The figure shows three views and two pictorial views of one solid part (mm, origin at its lowest corner). Answer the questions. A direction names the side the tool comes from. Coordinates: 2 decimals unless noted, no trailing zeros. Loops run counter-clockwise (first coordinate to the right, second up) from the corner with the lowest first, then second, coordinate; pieces in that order, holes last.
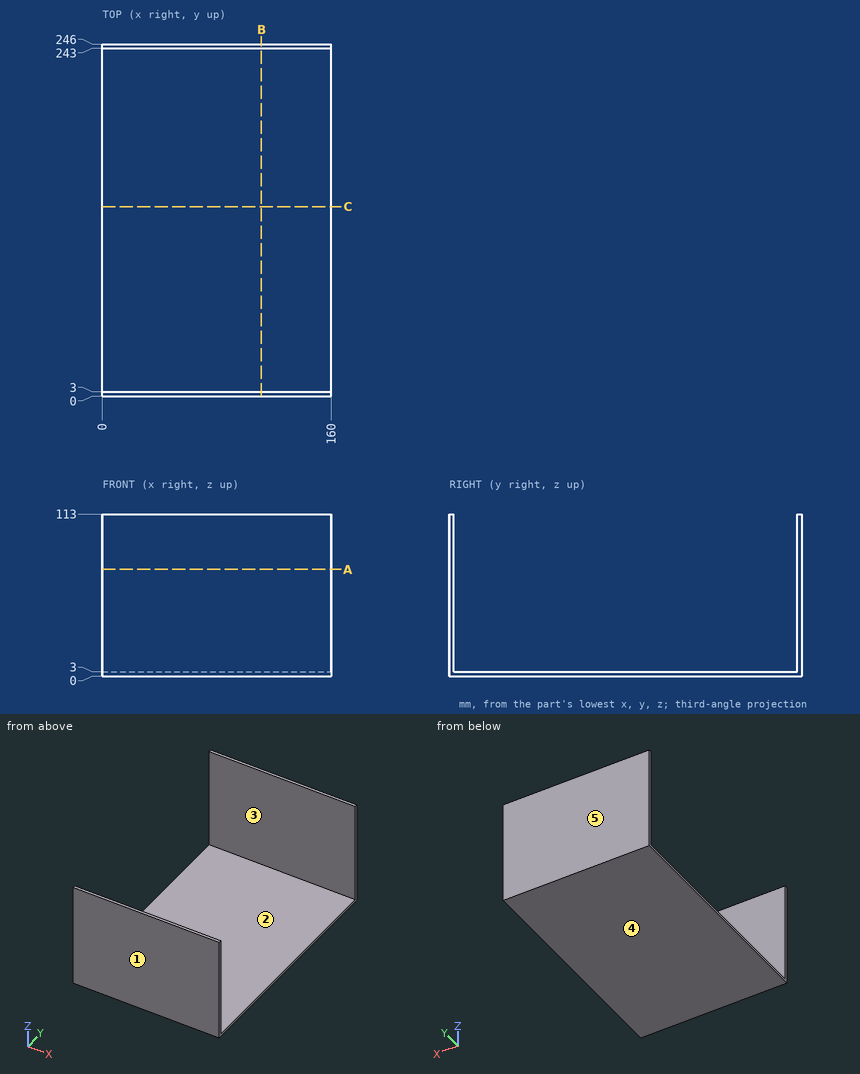
1. For the marked faces 1 and 2, determine the directions among +Z, -Z, +X, -X, +Y, -Y from which every point of the face is accessible in a straight line to the end or side of a thin tool.
2. A cutting plane is placed at A-A, the plane z = 74.5. Give the vertices of the cut face in (x, y), then the cut area to 3 significant figures.
3. Each of these flat-tipped pins is pushed along its axis until it touches: P1, Ø3, axis at x = 113, z = 70, coming from the -Y side; P2, Ø1, axis at x = 87.5, y = 116, coming from the +Z side. Where does it stop, or does it pass through?
4. A cutting plane is placed at C-C, the plane y = 132.5. Give the vertices of the cut face in (x, z).
5. Determine the mould class of the marked faces 3, 4 and 5 for opening direction Y: released by +Y, released by -Y, zero draft, split by the parting line, or undercut.
6. A cutting plane is placed at B-B, the plane x = 111. Give the vertices of the cut face in (y, z), then the cut area to 3 significant figures.
7. Straight lines are drawn through the part: probe 1 along Y at (x, z) = (88, 13); probe 2 along Z at (x, y) = (67, 230). For each, find the intervals that lie inside material, in ascending order.
Answers below:
1. face 1: +Z, -Z, +X, -X, -Y
1. face 2: +Z, +X, -X
2. outline: (0, 0) - (160, 0) - (160, 3) - (0, 3) - close; (0, 243) - (160, 243) - (160, 246) - (0, 246) - close
2. area: 960 mm2
3. P1: stops at y = 0
3. P2: stops at z = 3
4. outline: (0, 0) - (160, 0) - (160, 3) - (0, 3) - close
5. face 3: undercut
5. face 4: zero draft
5. face 5: released by +Y
6. outline: (0, 0) - (246, 0) - (246, 113) - (243, 113) - (243, 3) - (3, 3) - (3, 113) - (0, 113) - close
6. area: 1,400 mm2
7. probe 1: y = 0 to 3, 243 to 246
7. probe 2: z = 0 to 3
